Geometry: final body of the model. Coordinates: model frame, mm. A direction names the side the tool comes from. Round coordinates to 2 decimals unless told otherwise and drop trailing zeros. Write each loop counter-clockwise with the first axis right and the second up, starting at its lowest first coordinate (ties: lowest second). Pieces come first, ordered by that corner, then holes. Notation, with made-up numbers: M 33.5,-25.75 L 50.5,-25.75 A18 ccw 50.5,6.25 Z; hole C 39.25,-23 d5. An arc over 180 degrees is marked long. Use one line per item in the form item = value. Start each with the question number.
Item 1: Section query B-B (y = 22). Return loops of the section in (x, z), and give its area (3 significant figures).
Item 2: Section query D-D (y = 4). Return loops of the section in (x, z), and give its area (3 significant figures).
Item 3: Pin query (flat end, axial travel): pin 1 Ø19 at (x, z) = (34.45, 25) entering from +Y; pin 2 Ø5 at (y, z) = (5, 16) entering from -X; pin 3 Ø6 at (y, z) = (30, -2.5) entering from -X. Return the tip coordinate at first contact, or that it passes through.
Item 4: Section query C-C (z = 28.5). Return loops of the section in (x, y).
Item 5: Section query A-A (z = 0). Return loops of the section in (x, y).
Item 6: Pull-direction query (Y, two-part tool) for faces 1 (the cylindrical face through (-48.37, 28.76, -0.11)), 2 (the cylindrical face through (-59.91, 33.24, 0.11)), 3 (the flat face through (-31, 17, -8)); classes: pulls with the +Y half, pulls with the -Y half, needs draft (parallel to the pull), parting line crosses it, or undercut.
Item 7: Reachability of faces 4 (the flat face through (16.446, 5, 16)), 5 (the flat face through (16.446, 5, -17)), 6 (the cylindrical face through (-3.83, 16.13, 0.11)) from +Z, -Z, +X, -X, +Y, -Y: full face, straight path, thin tool, end or side. Return the list, or none.
Item 8: Ray query, probe 1 along Z at (x, y) = (-21, 19); probe 2 along X at (y, z) = (3.75, 0); probe 3 along X at (y, z) = (24, 3.5). Return the intervals inside material, ascending.
from build123d import *

# Parameters (mm, degrees)
ARM_PROFILE_SKETCH_R     = 10
ARM_BODY_DEPTH           = 8
MOUNTING_FLANGE_SKETCH_R = 6
MOUNTING_FLANGE_DEPTH    = 10
TRIM_CUT_SKETCH_R        = 6
TRIM_CUT_DEPTH           = 117.189881419


with BuildPart() as part:
    # Arm Profile Sketch → Arm Body (new, symmetric)
    with BuildSketch(Plane.XY):
        with BuildLine():
            Line((-41, 0), (86, 0))
            Line((86, 0), (86, 10))
            Line((86, 10), (20.155539406, 10))
            ThreePointArc((20.155539406, 10), (-4.14009349, 16.299631326), (-22.313585182, 33.611111111))
            ThreePointArc((-22.313585182, 33.611111111), (-60.228162216, 32.690078474), (-41, 0))
        make_face()
        with Locations((-41, 22)):
            Circle(ARM_PROFILE_SKETCH_R, mode=Mode.SUBTRACT)
    extrude(amount=ARM_BODY_DEPTH, both=True)

    # Mounting Flange Sketch → Mounting Flange (add)
    with BuildSketch(Plane(origin=(0, 10, 0), x_dir=(1, 0, 0), z_dir=(0, 1, 0))):
        with BuildLine():
            Line((16.445539406, 25), (16.445539406, -25))
            ThreePointArc((16.445539406, -25), (28.412643024, -41.958896227), (48.401557323, -36.367918187))
            ThreePointArc((48.401557323, -36.367918187), (64.807593984, -23.224109156), (85.166263205, -17.985565246))
            ThreePointArc((85.166263205, -17.985565246), (102.445539406, 0), (85.166263205, 17.985565246))
            ThreePointArc((85.166263205, 17.985565246), (64.807593984, 23.224109156), (48.401557323, 36.367918187))
            ThreePointArc((48.401557323, 36.367918187), (28.412643024, 41.958896227), (16.445539406, 25))
        make_face()
        with Locations((84.445539406, 0)):
            Circle(MOUNTING_FLANGE_SKETCH_R, mode=Mode.SUBTRACT)
        with Locations(Location((34.445539406, 25, 0), (0, 0, 270))):
            Circle(MOUNTING_FLANGE_SKETCH_R, mode=Mode.SUBTRACT)
        with Locations(Location((34.445539406, -25, 0), (0, 0, 270))):
            Circle(MOUNTING_FLANGE_SKETCH_R, mode=Mode.SUBTRACT)
    extrude(amount=-MOUNTING_FLANGE_DEPTH)

    # Trim Cut Sketch → Trim Cut (cut, through all)
    with BuildSketch(Plane(origin=(0, 10, 0), x_dir=(1, 0, 0), z_dir=(0, 1, 0))):
        with Locations(Location((84.445539406, 0, 0), (0, 0, 270))):
            Circle(TRIM_CUT_SKETCH_R)
    extrude(amount=-TRIM_CUT_DEPTH, mode=Mode.SUBTRACT)


solid = part.part
Working result:
q1.outline = M -63,-8 L -51,-8 L -51,8 L -63,8 Z; M -31,-8 L -12.34,-8 L -12.34,8 L -31,8 Z
q1.area = 491 mm²
q2.outline = M -53.65,-8 L 16.45,-8 L 16.45,-25 A18 ccw 48.4,-36.37 A50 cw 85.17,-17.99 A18 ccw 85.17,17.99 A50 cw 48.4,36.37 A18 ccw 16.45,25 L 16.45,8 L -53.65,8 Z; hole C 34.45,-25 d12; hole C 34.45,25 d12; hole C 84.45,0 d12
q2.area = 5,570 mm²
q3.pin_1 = 10
q3.pin_2 = 16.45
q3.pin_3 = -62.42
q4.outline = M 16.79,0 L 29.57,0 L 29.57,10 L 16.79,10 Z; M 39.32,0 L 56.44,0 L 56.44,10 L 39.32,10 Z
q5.outline = M -41,0 L 78.45,0 L 78.45,10 L 20.16,10 A50 cw -22.31,33.61 A22 ccw long Z; M 90.45,0 L 102.45,0 L 102.45,10 L 90.45,10 Z; hole C -41,22 d20
q6.face_1 = undercut
q6.face_2 = parting line crosses it
q6.face_3 = needs draft
q7.face_4 = +Z, -X, +Y, -Y
q7.face_5 = -Z, -X, +Y, -Y
q7.face_6 = +Z, -Z, +X, +Y
q8.probe_1 = -8 to 8
q8.probe_2 = -53.29 to 78.45, 90.45 to 102.45
q8.probe_3 = -62.91 to -50.8, -31.2 to -14.54
